Work out the finished part from the listing and answer in its coordinate system (mm). A direction names the side the tool comes from. Coordinates: 2 decimals unless noted, no trailing zeros. Order: outer loops, then holes, each group sorted by start corner. A loop starts at its lowest first (then second) coordinate and runs counter-clockwise, first axis right, second up. Notation, with made-up numbers: (-26, 47.25) -> (-10, 47.25) arc R25 ccw to (-10, 75.25) -> close; hole circle Ø6 at (-16, 59). An arc over 180 degrees is marked (long way). Write item = value, one per line. Start each with the question number.
Q1. The part is cut by section D-D, the plane y = 107.5. Determine the outline of the cut face in (x, z).
Q2. The part is cut by section A-A, the plane x = 37. Determine the outline of the cut face in (y, z), plus the area to 3 significant figures.
Q3. The part is cut by section C-C, the plane x = 0. Determine the outline of the cut face in (y, z), plus the area to 3 significant figures.
Q4. The part is cut by section B-B, the plane z = 0. Determine the outline of the cut face in (x, y), plus the area to 3 significant figures.
Q5. Which of the six approach directions +Z, -Z, +X, -X, +Y, -Y give full straight-line access (tool end or side, diameter ignored) to faces 5 (the flat face through (4, 91, -4)), 6 (the flat face through (0, 131, 0))?
Q6. Straight lines are drawn through the part: L1, parallel to Z at x = 37, y = 2; L2, parallel to Y at x = 26, z = -20.5; L3, parallel to X at y = 19, z = 0. For each, find the intervals that lie inside material, in ascending order. Write a range as from..to.
Q7. Flat-ended cylindrical pins translate along their axes: pin 1 (1.5 mm diameter, centred on x = 2.5, y = 24.5, fed in from +Z); pin 2 (6 mm diameter, centred on y = 39.5, z = 8.5, fed in from -X); pin 3 (2 mm diameter, centred on x = -21.5, z = -3, fed in from +Y). Find the tip coordinate at first contact, or state that the pin passes through.
Q8. For a pull along Z with two mould halves and no side action, classify faces 1 (the cylindrical face through (-41.292, 2.958, -1.352)), 2 (the flat face through (-1, 3, -27.5)), 3 (the cylindrical face through (32.708, 2.958, -1.352)), 4 (the flat face through (44, 3, 0)) as +Z half, -Z half, draft (parallel to the pull), parting line (faces both ways), or undercut.
```python
from build123d import *

# Parameters (mm, degrees)
SKETCH_1_W         = 88
SKETCH_1_H         = 55
EXTRUDE_1_DEPTH    = 6
HOLE_WIZARD_M8_1_D = 9
SKETCH_4_R         = 20
EXTRUDE_2_DEPTH    = 85
SKETCH_5_R         = 5
EXTRUDE_3_DEPTH    = 40


with BuildPart() as part:
    # 草图1 → 凸台-拉伸1 (new body)
    with BuildSketch(Plane(origin=(0, 0, 0), x_dir=(1, 0, 0), z_dir=(0, 1, 0))):
        Rectangle(SKETCH_1_W, SKETCH_1_H)
    extrude(amount=EXTRUDE_1_DEPTH)

    # M8 间隙孔1 (through all)
    with Locations(Plane(origin=(0, 6, 0), x_dir=(1, 0, 0), z_dir=(0, 1, 0))):
        with Locations((-37, 0), (37, 0)):
            Hole(HOLE_WIZARD_M8_1_D / 2)

    # 草图4 → 凸台-拉伸2 (add)
    with BuildSketch(Plane(origin=(0, 6, 0), x_dir=(1, 0, 0), z_dir=(0, 1, 0))):
        with Locations(Location((0, 0, 0), (0, 0, 90))):
            Circle(SKETCH_4_R)
    extrude(amount=EXTRUDE_2_DEPTH)

    # 草图5 → 凸台-拉伸3 (add)
    with BuildSketch(Plane(origin=(0, 91, 0), x_dir=(1, 0, 0), z_dir=(0, 1, 0))):
        with Locations(Location((0, 0, 0), (0, 0, 270))):
            Circle(SKETCH_5_R)
    extrude(amount=EXTRUDE_3_DEPTH)


solid = part.part
```
Model answer:
q1.outline = circle Ø10 at (0, 0)
q2.outline = (0, -27.5) -> (6, -27.5) -> (6, -4.5) -> (0, -4.5) -> close; (0, 4.5) -> (6, 4.5) -> (6, 27.5) -> (0, 27.5) -> close
q2.area = 276 mm2
q3.outline = (0, -27.5) -> (6, -27.5) -> (6, -20) -> (91, -20) -> (91, -5) -> (131, -5) -> (131, 5) -> (91, 5) -> (91, 20) -> (6, 20) -> (6, 27.5) -> (0, 27.5) -> close
q3.area = 4,130 mm2
q4.outline = (-44, 0) -> (-41.5, 0) -> (-41.5, 6) -> (-44, 6) -> close; (-32.5, 0) -> (32.5, 0) -> (32.5, 6) -> (20, 6) -> (20, 91) -> (5, 91) -> (5, 131) -> (-5, 131) -> (-5, 91) -> (-20, 91) -> (-20, 6) -> (-32.5, 6) -> close; (41.5, 0) -> (44, 0) -> (44, 6) -> (41.5, 6) -> close
q4.area = 4,220 mm2
q5.face_5 = +Y
q5.face_6 = +Z, -Z, +X, -X, +Y
q6.L1 = -27.5..-4.5, 4.5..27.5
q6.L2 = 0..6
q6.L3 = -20..20
q7.pin_1 = 19.92
q7.pin_2 = -19.23
q7.pin_3 = 6
q8.face_1 = undercut
q8.face_2 = -Z half
q8.face_3 = undercut
q8.face_4 = draft
